Source: CAD feature listing. Evaluate the final solid. Frame: model axes, mm. Coordinates: 2 decimals unless noted, no trailing zeros. Write each loop counter-clockwise with the first axis right and the second up, starting at its lowest first coordinate (ties: lowest second). Pieces come first, ordered by that corner, then holes. Notation, with made-up numbers: (70.25, 81.25) -> (103.25, 81.25) arc R26 cw to (103.25, 112.25) -> close; hole circle Ø9 at (51, -27.75). An arc over 180 degrees is marked (long way). One line per item, written item: value. Start each with the question number.
1. Section query B-B, the plane z = 0.15. Output: boundary loops of the cut face in (x, y), and give its area (3 significant figures).
2. Section query A-A, the plane x = 0.5. Output: boundary loops of the cut face in (y, z).
3. Mould query, pull axis Y, two halves, no side actions, for faces 1 (the flat face through (0.1, 0.7, -0.5)), 2 (the cylindrical face through (8.5, 0, 0)), 3 (the cylindrical face through (0.428, 0.545, -0.007)). Classes: released by +Y, released by -Y, zero draft, split by the parting line, or undercut.
4. Line query: line 1 (X direction, y = 0.05, z = 0.3); line 2 (X direction, y = -0.35, z = 0.1); line 3 (Y direction, x = -7.5, z = 0.25). Output: solid intervals per line, ascending.
5. Section query C-C, the plane y = -0.3. Output: boundary loops of the cut face in (x, z), and give its area (3 significant figures).
from build123d import *

# Parameters (mm, degrees)
SKETCH1_R           = 0.55
THIGH1_LENGTH_DEPTH = 0.5


with BuildPart() as part:
    # Sketch1 → Thigh1 length (new, symmetric)
    with BuildSketch(Plane.XY):
        with BuildLine():
            Line((-7.5, 1), (7.5, 1))
            ThreePointArc((7.5, 1), (8.5, 0), (7.5, -1))
            Line((7.5, -1), (-7.5, -1))
            ThreePointArc((-7.5, -1), (-8.5, 0), (-7.5, 1))
        make_face()
        with Locations((-7.5, 0)):
            Circle(SKETCH1_R, mode=Mode.SUBTRACT)
        with Locations((7.5, 0)):
            Circle(SKETCH1_R, mode=Mode.SUBTRACT)
        with Locations((0.5, 0)):
            Circle(SKETCH1_R, mode=Mode.SUBTRACT)
    extrude(amount=THIGH1_LENGTH_DEPTH, both=True)


solid = part.part
Computed values:
1. outline: (-7.5, -1) -> (7.5, -1) arc R1 ccw to (7.5, 1) -> (-7.5, 1) arc R1 ccw to start; hole circle Ø1.1 at (-7.5, 0); hole circle Ø1.1 at (0.5, 0); hole circle Ø1.1 at (7.5, 0)
1. area: 30.3 mm²
2. outline: (-1, -0.5) -> (-0.55, -0.5) -> (-0.55, 0.5) -> (-1, 0.5) -> close; (0.55, -0.5) -> (1, -0.5) -> (1, 0.5) -> (0.55, 0.5) -> close
3. face 1: zero draft
3. face 2: split by the parting line
3. face 3: undercut
4. line 1: x = -8.5 to -8.05, -6.95 to -0.05, 1.05 to 6.95, 8.05 to 8.5
4. line 2: x = -8.44 to -7.92, -7.08 to 0.08, 0.92 to 7.08, 7.92 to 8.44
4. line 3: y = -1 to -0.55, 0.55 to 1
5. outline: (-8.45, -0.5) -> (-7.96, -0.5) -> (-7.96, 0.5) -> (-8.45, 0.5) -> close; (-7.04, -0.5) -> (0.04, -0.5) -> (0.04, 0.5) -> (-7.04, 0.5) -> close; (0.96, -0.5) -> (7.04, -0.5) -> (7.04, 0.5) -> (0.96, 0.5) -> close; (7.96, -0.5) -> (8.45, -0.5) -> (8.45, 0.5) -> (7.96, 0.5) -> close
5. area: 14.1 mm²
